Part print with two shaded views. Sizes in mm from the minimum x, y, z corner. Coordinates: 2 decimals unless noted, no trailing zeros. Write each loop counter-clockwise with the first axis right and the second up, starting at its lowest first coordinate (ties: lowest second). Pieces come first, ordered by that corner, then holes.
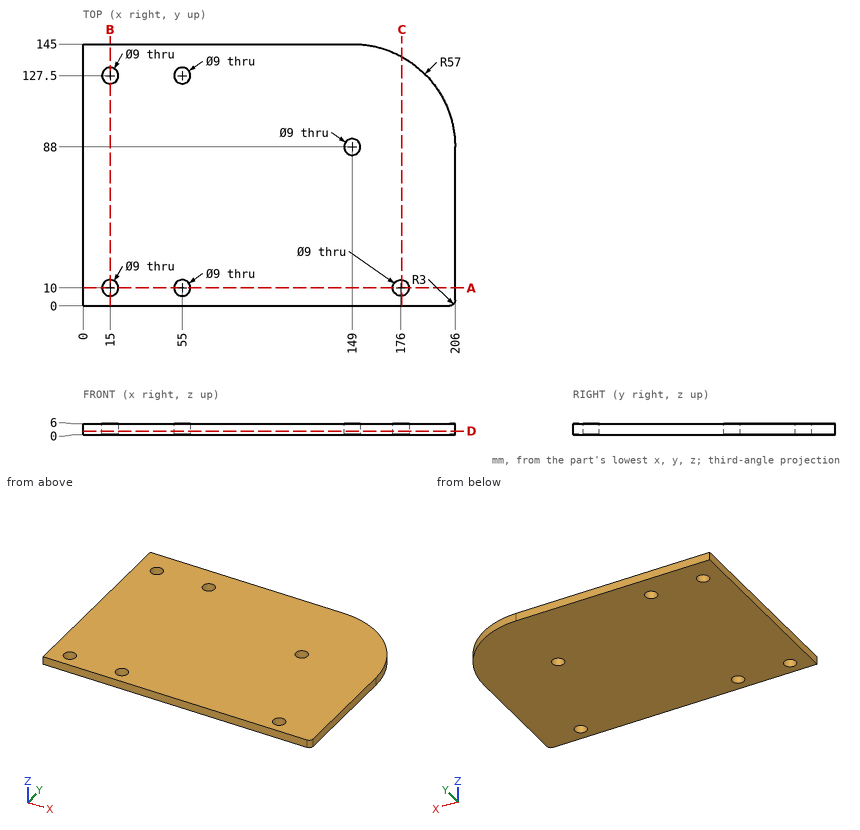
(1) Slice it at D-D, the plane z = 2. List the corners of the cut face in (x, y).
(2) Slice it at B-B, the plane x = 15. List the corners of the cut face in (y, z).
(3) Slice it at A-A, the plane y = 10. List the corners of the cut face in (x, z), and give its area (3 significant figures).
(4) Probe L1, parallel to Y at x = 15, z = 3.85; L2, parallel to X at y = 10.5, z = 4.5; L3, parallel to Y at x = 58, z = 1.05. List the from-to ranges inside material, lowest first.
(5) Slice it at C-C, the plane x = 176.5. List the corners of the cut face in (y, z).
Results:
1. outline: (0, 0) - (203, 0) arc R3 ccw to (206, 3) - (206, 88) arc R57 ccw to (149, 145) - (0, 145) - close; hole circle Ø9 at (15, 10); hole circle Ø9 at (15, 127.5); hole circle Ø9 at (55, 10); hole circle Ø9 at (55, 127.5); hole circle Ø9 at (149, 88); hole circle Ø9 at (176, 10)
2. outline: (0, 0) - (5.5, 0) - (5.5, 6) - (0, 6) - close; (14.5, 0) - (123, 0) - (123, 6) - (14.5, 6) - close; (132, 0) - (145, 0) - (145, 6) - (132, 6) - close
3. outline: (0, 0) - (10.5, 0) - (10.5, 6) - (0, 6) - close; (19.5, 0) - (50.5, 0) - (50.5, 6) - (19.5, 6) - close; (59.5, 0) - (171.5, 0) - (171.5, 6) - (59.5, 6) - close; (180.5, 0) - (206, 0) - (206, 6) - (180.5, 6) - close
3. area: 1,070 mm2
4. L1: y = 0 to 5.5, 14.5 to 123, 132 to 145
4. L2: x = 0 to 10.53, 19.47 to 50.53, 59.47 to 171.53, 180.47 to 206
4. L3: y = 0 to 6.65, 13.35 to 124.15, 130.85 to 145
5. outline: (0, 0) - (5.53, 0) - (5.53, 6) - (0, 6) - close; (14.47, 0) - (137.93, 0) - (137.93, 6) - (14.47, 6) - close
